Answer from the drawing. Dimensions are ordinates in mm from the lowest x, y and z of the part. Coordinates: 2 decimals unless noted, no trailing zeros. Order: outer loops, then holes, each group sorted by start corner. A loop starts at its lowest first (then second) coordinate and runs counter-clockwise, first axis right, second up. Notation, with made-up numbers: (33, 55) - (54, 55) arc R31 ccw to (54, 82) - close; hole circle Ø3 at (71, 9). An arc over 180 degrees is marked (long way). Use a Markdown table: item, result. Add a question column.
Item 1: The mould has two halves that part along Y. Classify the marked faces 1, 2, 3 and 4: released by +Y, released by -Y, zero draft, split by the parting line, or undercut.
Item 2: The part is cut by section D-D, the plane y = 3.75. Give the vertices of the cut face in (x, z) (1 decimal), then the cut area to 3 significant figures.
Item 3: The part is cut by section A-A, the plane x = 12. Give the vertices of the cut face in (y, z) (1 decimal), then the cut area to 3 significant figures.
Item 4: Flat-ended cylindrical pins translate along their axes: P1, Ø2, axis at x = 17, y = 9.5, coming from the -Z side; P2, Ø2, axis at y = 8, z = 5, coming from the +X side; P3, Ø2, axis at y = 8, z = 8.5, coming from the -X side. Find the tip coordinate at first contact, or state that the pin passes through.
Item 5: Find the intervals of material crossed by line 1 along Y through (x, z) = (12, 7.75) (1 decimal); line 2 along X through (y, z) = (6, 6.5) (1 decimal); line 3 along Y through (x, z) = (8, 11) (1 decimal), in increasing order.
Item 6: The part is cut by section B-B, the plane z = 2.25. Give the vertices of the cut face in (x, y) (1 decimal).
Item 7: The part is cut by section C-C, the plane x = 16.5. Give the vertices of the cut face in (y, z) (1 decimal).
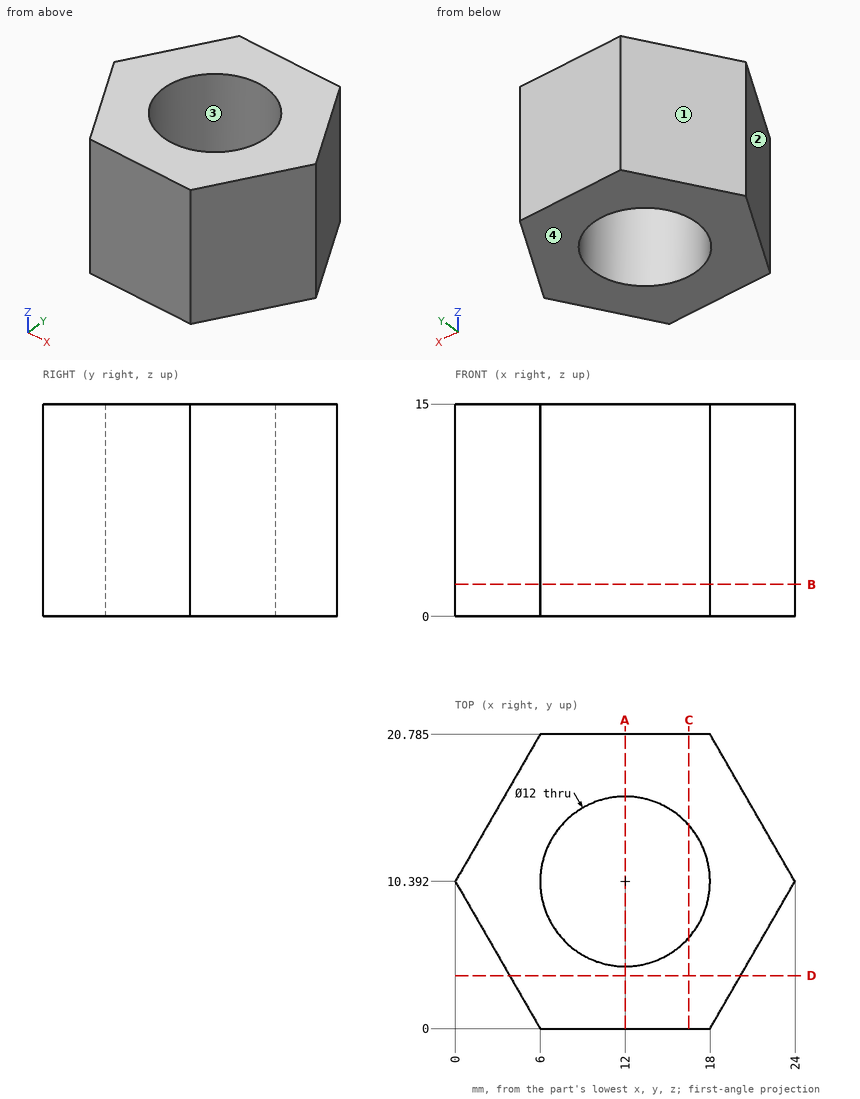
Solution:
| question | item | result |
|---|---|---|
| 1 | face 1 | released by +Y |
| 1 | face 2 | released by -Y |
| 1 | face 3 | undercut |
| 1 | face 4 | zero draft |
| 2 | outline | (3.8, 0) - (20.2, 0) - (20.2, 15) - (3.8, 15) - close |
| 2 | area | 245 mm2 |
| 3 | outline | (0, 0) - (4.4, 0) - (4.4, 15) - (0, 15) - close; (16.4, 0) - (20.8, 0) - (20.8, 15) - (16.4, 15) - close |
| 3 | area | 132 mm2 |
| 4 | P1 | stops at z = 0 |
| 4 | P2 | stops at x = 23.2 |
| 4 | P3 | stops at x = 0.8 |
| 5 | line 1 | y = 0 to 4.4, 16.4 to 20.8 |
| 5 | line 2 | x = 2.5 to 7.9, 16.1 to 21.5 |
| 5 | line 3 | y = 0 to 5.9, 14.9 to 20.8 |
| 6 | outline | (0, 10.4) - (6, 0) - (18, 0) - (24, 10.4) - (18, 20.8) - (6, 20.8) - close; hole circle Ø12 at (12, 10.4) |
| 7 | outline | (0, 0) - (6.4, 0) - (6.4, 15) - (0, 15) - close; (14.4, 0) - (20.8, 0) - (20.8, 15) - (14.4, 15) - close |
